The model under review builds one solid part; all positions refer to its coordinate system, in mm. Round coordinates to 2 decimals unless told otherwise and drop trailing zeros. Loops run counter-clockwise (first coordinate to the right, second up) from the corner with the lowest first, then second, coordinate; pieces in that order, holes last. Notation, with made-up numbers: (-39, 41) -> (8, 41) arc R28 ccw to (8, 80) -> close; hole circle Ø7 at (-32.5, -21.5). An arc over 180 degrees is marked (long way). Write each question's results on one line, items separated by ' | '. Start each with the question number.
Item 1: We need section B-B (x = -365). Give the boundary of the cut face in (y, z), and give its area (3 significant figures).
Item 2: We need section C-C (y = 330). Give the boundary of the cut face in (x, z).
Item 3: We need section A-A (y = 80). Give the boundary of the cut face in (x, z), and give its area (3 significant figures).
Item 4: We need section D-D (z = 13.25). Give the number of separate pieces and of enclosed holes in the cut face, and give its area (3 significant figures).
Item 5: For L1, parallel to Y at x = -365, z = 7; L2, parallel to Y at x = 0, z = 9.25; L3, parallel to X at y = -172, z = 10.5, list the stretches that pass through material, from the lowest coordinate up. Write a range as from..to.
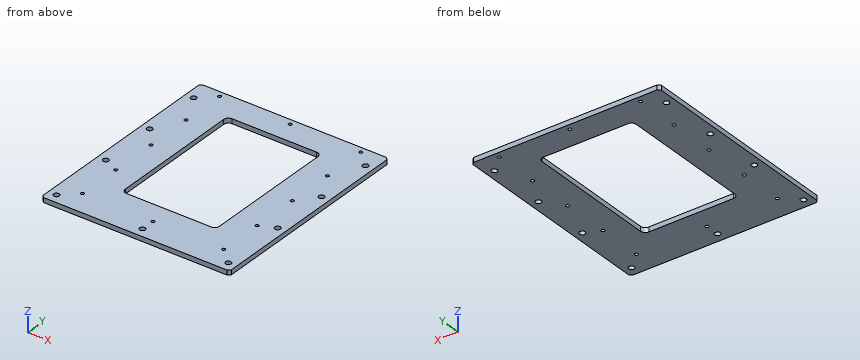
from build123d import *

# Parameters (mm, degrees)
SKETCH_1_W              = 800
SKETCH_1_H              = 980
EXTRUDE_1_DEPTH         = 20
HOLE_WIZARD_M16_1_D     = 14
HOLE_WIZARD_M16_1_DEPTH = 42
HOLE_WIZARD_M16_1_TIP   = 4.206024333
SKETCH_4_W              = 400
SKETCH_4_H              = 600
CUT_EXTRUDE_1_DEPTH     = 20
FILLET_1_R              = 20
SKETCH_10_W             = 800
SKETCH_10_H             = 75
CUT_EXTRUDE_3_DEPTH     = 633.850693292
HOLE_WIZARD_24_0_24_1_D = 24
CHAMFER_1_SIZE          = 10


with BuildPart() as part:
    # 草图1 → 凸台-拉伸1 (new body)
    with BuildSketch(Plane.XY):
        Rectangle(SKETCH_1_W, SKETCH_1_H)
    extrude(amount=EXTRUDE_1_DEPTH)

    # M16 螺纹孔1
    with Locations(Plane.XY.offset(20)):
        with Locations((300, 390), (-300, -390), (-300, 390), (300, -390), (-300, 0), (0, -390), (300, 0), (0, 390), (-300, 200), (300, 200), (-300, -200), (300, -200)):
            Hole(HOLE_WIZARD_M16_1_D / 2, depth=HOLE_WIZARD_M16_1_DEPTH)
            with Locations((0, 0, -(HOLE_WIZARD_M16_1_DEPTH + HOLE_WIZARD_M16_1_TIP / 2))):  # 118° drill point
                Cone(0, HOLE_WIZARD_M16_1_D / 2, HOLE_WIZARD_M16_1_TIP, mode=Mode.SUBTRACT)

    # 草图4 → 切除-拉伸1 (cut)
    with BuildSketch(Plane.XY.offset(20)):
        Rectangle(SKETCH_4_W, SKETCH_4_H)
    extrude(amount=-CUT_EXTRUDE_1_DEPTH, mode=Mode.SUBTRACT)

    # 圆角1
    fillet_1_edges = [part.edges().sort_by_distance(p)[0] for p in [
        (200, 300, 10),
        (200, -300, 10),
        (-200, -300, 10),
        (-200, 300, 10),
    ]]
    fillet(fillet_1_edges, radius=FILLET_1_R)

    # 草图10 → 切除-拉伸3 (cut, through all)
    with BuildSketch(Plane.XY.offset(20)):
        with Locations((0, 452.5)):
            Rectangle(SKETCH_10_W, SKETCH_10_H)
    extrude(amount=-CUT_EXTRUDE_3_DEPTH, mode=Mode.SUBTRACT)

    # Ø24.0 (24) 直径孔1 (through all)
    with Locations(Plane.XY.offset(20)):
        with Locations((365, 80), (365, -450), (-365, -450), (0, -450), (0, 450), (-365, 330), (365, 330), (-365, 80), (-365, -170), (365, -170)):
            Hole(HOLE_WIZARD_24_0_24_1_D / 2)

    # 倒角1
    chamfer_1_edges = [part.edges().sort_by_distance(p)[0] for p in [
        (-400, 415, 10),
        (400, 415, 10),
        (400, -490, 10),
        (-400, -490, 10),
    ]]
    chamfer(chamfer_1_edges, length=CHAMFER_1_SIZE)


solid = part.part
Here are the results:
1) outline: (-490, 0) -> (-462, 0) -> (-462, 20) -> (-490, 20) -> close; (-438, 0) -> (-182, 0) -> (-182, 20) -> (-438, 20) -> close; (-158, 0) -> (68, 0) -> (68, 20) -> (-158, 20) -> close; (92, 0) -> (318, 0) -> (318, 20) -> (92, 20) -> close; (342, 0) -> (415, 0) -> (415, 20) -> (342, 20) -> close | area: 16,200 mm2
2) outline: (-400, 0) -> (-377, 0) -> (-377, 20) -> (-400, 20) -> close; (-353, 0) -> (353, 0) -> (353, 20) -> (-353, 20) -> close; (377, 0) -> (400, 0) -> (400, 20) -> (377, 20) -> close
3) outline: (-400, 0) -> (-377, 0) -> (-377, 20) -> (-400, 20) -> close; (-353, 0) -> (-200, 0) -> (-200, 20) -> (-353, 20) -> close; (200, 0) -> (353, 0) -> (353, 20) -> (200, 20) -> close; (377, 0) -> (400, 0) -> (400, 20) -> (377, 20) -> close | area: 7,040 mm2
4) separate pieces: 1 | enclosed holes: 22 | area: 478,000 mm2
5) L1: y = -490..-462, -438..-182, -158..68, 92..318, 342..415 | L2: y = -490..-462, -438..-397, -383..-300, 300..383, 397..415 | L3: x = -400..-376.83, -353.17..-200, 200..353.17, 376.83..400
